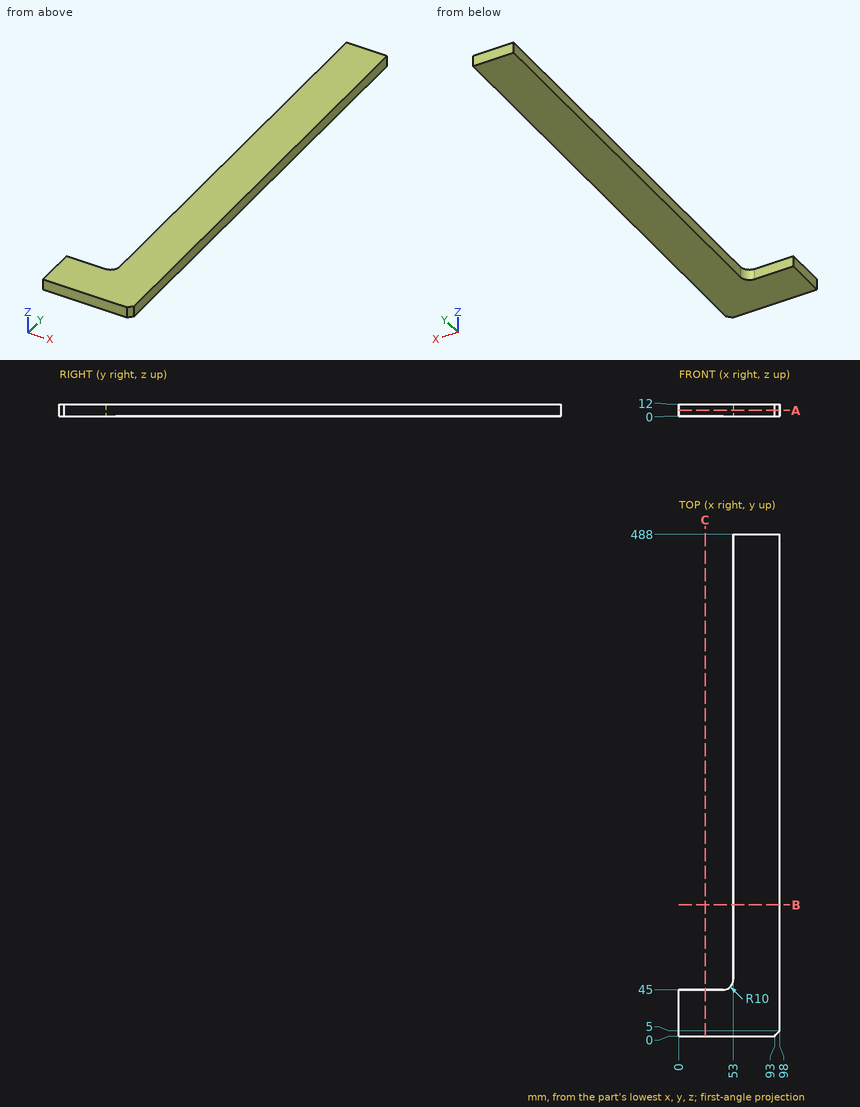
Could you check a few things on this drawing? It's one solid part, dimensions in mm from its lowest x, y, z. Coordinates: 2 decimals unless noted, no trailing zeros. Order: outer loops, then holes, each group sorted by start corner. A loop starts at its lowest first (then second) coordinate and runs counter-clockwise, first axis right, second up. Notation, with made-up numbers: M 81.5,52.25 L 99.5,52.25 A22 cw 99.5,75.25 Z; hole C 28,82.5 d11. An arc over 180 degrees is marked long. Use one line per item in the form item = value. Start each with the question number.
1. Suppose I cut it at B-B on y = 127.5. Write out the boundary of the cut face in (x, z).
2. Please list where these lines run through material, in increasing order: line 1 (X direction, y = 329.5, z = 10.5); line 2 (Y direction, x = 27, z = 8.5); line 3 (Y direction, x = 46, z = 6.75).
3. For pin 1 (6 mm diameter, centred on x = 18.5, z = 1.5, fed in from -Y); pin 2 (6 mm diameter, centred on y = 331.5, z = 6, fed in from -X); pin 3 (3.5 mm diameter, centred on x = 11.5, z = 7.5, fed in from +Y), each with a flat end and sliding along its axis, tell me the tip position at first contact or that it passes through.
4. Suppose I cut it at C-C on x = 25.5. Write out the boundary of the cut face in (y, z).
5. Suppose I cut it at A-A on z = 5.75. Write out the boundary of the cut face in (x, y), then the cut area to 3 significant figures.
Geometry says:
q1.outline = M 53,0 L 98,0 L 98,12 L 53,12 Z
q2.line_1 = 53 to 98
q2.line_2 = 0 to 45
q2.line_3 = 0 to 45.46
q3.pin_1 = 0
q3.pin_2 = 53
q3.pin_3 = 45
q4.outline = M 0,0 L 45,0 L 45,12 L 0,12 Z
q5.outline = M 0,0 L 93,0 L 98,5 L 98,488 L 53,488 L 53,55 A10 cw 43,45 L 0,45 Z
q5.area = 24,400 mm^2
